For this review, take the finished solid that the model builds, in its own axes (mm). Give positions to 0.01 mm unless a question says otherwise; leave off trailing zeros. Loops run counter-clockwise (first coordinate to the right, second up) from the corner with the lowest first, then second, coordinate; pieces in that order, holes last. Notation, with made-up numbers: (3.5, -30.5) -> (52.5, -30.5) arc R9 cw to (52.5, -25.5) -> close; hole circle Ø6 at (-1.75, 53). An arc over 180 degrees is marked (long way). Write each question's results on one line, items separated by ' | '. Start each with the question number.
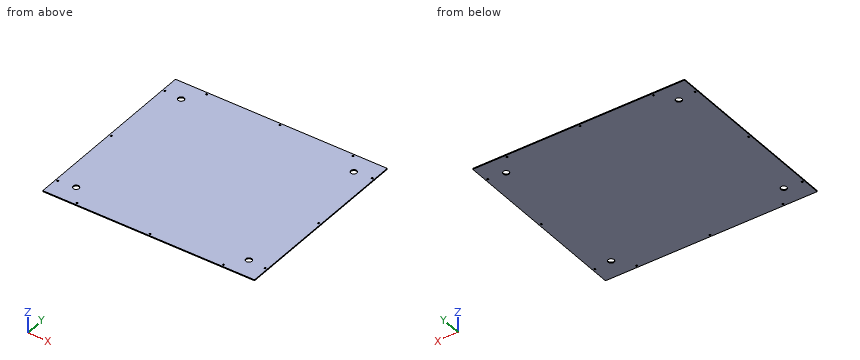
```python
from build123d import *

# Parameters (mm, degrees)
SKETCH_1_W               = 868
SKETCH_1_H               = 768
EXTRUDE_1_DEPTH          = 4
FILLET_1_R               = 2
HOLE_WIZARD_M6_1_D       = 7
HOLE_WIZARD_M6_2_D       = 7
CUT_EXTRUDE_1_REACH      = 581.507
SKETCH_7_R               = 12.5
MIRROR_5_COPY_1_REACH    = 581.507
MIRROR_5_COPY_1_SKETCH_R = 12.5


with BuildPart() as part:
    # 草图1 → 凸台-拉伸1 (new body)
    with BuildSketch(Plane.XY):
        Rectangle(SKETCH_1_W, SKETCH_1_H)
    extrude(amount=EXTRUDE_1_DEPTH)

    # 圆角1
    fillet_1_edges = [part.edges().sort_by_distance(p)[0] for p in [
        (-434, 384, 2),
        (434, 384, 2),
        (434, -384, 2),
        (-434, -384, 2),
    ]]
    fillet(fillet_1_edges, radius=FILLET_1_R)

    # M6 间隙孔1 (through all)
    with Locations(Plane.XY.offset(4)):
        with Locations((-425, 310), (-425, -310), (-425, 0)):
            hole_wizard_m6_1 = Hole(HOLE_WIZARD_M6_1_D / 2)

    # 镜向2: M6 间隙孔1 across plane
    add(hole_wizard_m6_1.mirror(Plane(origin=(0, 0, 0), x_dir=(0, 0, 1), z_dir=(1, 0, 0))), mode=Mode.SUBTRACT)

    # M6 间隙孔2 (through all)
    with Locations(Plane.XY.offset(4)):
        with Locations((-300, 375), (300, 375), (0, 375)):
            hole_wizard_m6_2 = Hole(HOLE_WIZARD_M6_2_D / 2)

    # 镜向3: M6 间隙孔2 across plane
    add(hole_wizard_m6_2.mirror(Plane.ZX), mode=Mode.SUBTRACT)

    # 草图7 → 切除-拉伸1 (cut, up to next)
    with BuildSketch(Plane.XY.offset(4), mode=Mode.PRIVATE) as cut_extrude_1_sk1:
        with Locations((-354, -304)):
            Circle(SKETCH_7_R)
    cut_extrude_1_tool1 = extrude(cut_extrude_1_sk1.sketch, amount=-CUT_EXTRUDE_1_REACH, mode=Mode.PRIVATE) & part.part
    cut_extrude_1 = cut_extrude_1_tool1.solids().sort_by_distance((-354, -304, 4))[0]
    add(cut_extrude_1, mode=Mode.SUBTRACT)

    # 镜向4: 切除-拉伸1 across plane
    add(cut_extrude_1.mirror(Plane(origin=(0, 0, 0), x_dir=(0, 0, 1), z_dir=(1, 0, 0))), mode=Mode.SUBTRACT)

    # 镜向5: 切除-拉伸1 across plane
    add(cut_extrude_1.mirror(Plane.ZX), mode=Mode.SUBTRACT)

    # 镜向5 copy 1 sketch → 镜向5 copy 1 (cut, up to next)
    with BuildSketch(Plane(origin=(0, 0, 4), x_dir=(-1, 0, 0), z_dir=(0, 0, 1)), mode=Mode.PRIVATE) as mirror_5_copy_1_sk1:
        with Locations((-354, -304)):
            Circle(MIRROR_5_COPY_1_SKETCH_R)
    mirror_5_copy_1_tool1 = extrude(mirror_5_copy_1_sk1.sketch, amount=-MIRROR_5_COPY_1_REACH, mode=Mode.PRIVATE) & part.part
    add(mirror_5_copy_1_tool1.solids().sort_by_distance((354, 304, 4))[0], mode=Mode.SUBTRACT)


solid = part.part
```
1. For pin 1 Ø9 at (x, y) = (-425, -310) entering from -Z; pin 2 Ø20 at (x, y) = (354, 304) entering from +Z, all flat-tipped, find the tip position at first contact; note any pin that passes through.
2. Wall thickness on L1, parallel to Y at x = 300, z = 2.4; L2, parallel to Y at x = 354, z = 2.3; L3, parallel to X at y = -375, z = 3.05: over which ranges is each line inside the solid? List them lowest first.
3. We need section A-A (x = -354). Write out the cut boundary in (y, z), plus the area to 3 significant figures.
Response:
1) pin 1: stops at z = 0 | pin 2: passes through
2) L1: y = -384 to -378.5, -371.5 to 371.5, 378.5 to 384 | L2: y = -384 to -316.5, -291.5 to 291.5, 316.5 to 384 | L3: x = -434 to -303.5, -296.5 to -3.5, 3.5 to 296.5, 303.5 to 434
3) outline: (-384, 0) -> (-316.5, 0) -> (-316.5, 4) -> (-384, 4) -> close; (-291.5, 0) -> (291.5, 0) -> (291.5, 4) -> (-291.5, 4) -> close; (316.5, 0) -> (384, 0) -> (384, 4) -> (316.5, 4) -> close | area: 2,870 mm2
